```python
from build123d import *

# Parameters (mm, degrees)
HEX_BODY_9AF_DEPTH            = 2.5
COLLAR_7_5_SKETCH_R           = 3.75
COLLAR_7_5_DEPTH              = 2
TIP_BODY_5_5_SKETCH_R         = 2.75
TIP_BODY_5_5_DEPTH            = 5
TIP_END_CHAMFER_0_5X30_SIZE   = 0.5
TIP_END_CHAMFER_0_5X30_SIZE2  = 0.288675135
TIP_BORE_2_5_SKETCH_R         = 1.25
TIP_BORE_2_5_DEPTH            = 4
SHANK_START                   = 3
SHANK_7_5_SKETCH_R            = 3.75
SHANK_7_5_DEPTH               = 3
SHANK_CHAMFER_1X45_SIZE       = 1
TERMINAL_NOTCH_CUT_DEPTH      = 12.7260394
TERMINAL_NOTCH_CUT_DEPTH_BACK = 12.7260394


with BuildPart() as part:
    # Hex Profile 9AF Sketch → Hex Body 9AF (new body)
    with BuildSketch(Plane.XY):
        Polygon((2.598076211, 4.5), (-2.598076211, 4.5), (-5.196152423, 0), (-2.598076211, -4.5), (2.598076211, -4.5), (5.196152423, 0), align=None)
    extrude(amount=HEX_BODY_9AF_DEPTH)

    # Collar Ø7.5 Sketch → Collar Ø7.5 (add)
    with BuildSketch(Plane.XY.offset(2.5)):
        Circle(COLLAR_7_5_SKETCH_R)
    extrude(amount=COLLAR_7_5_DEPTH)

    # Tip Body Ø5.5 Sketch → Tip Body Ø5.5 (add)
    with BuildSketch(Plane.XY.offset(4.5)):
        Circle(TIP_BODY_5_5_SKETCH_R)
    extrude(amount=TIP_BODY_5_5_DEPTH)

    # Tip End Chamfer 0.5x30
    tip_end_chamfer_0_5x30_edges = [part.edges().sort_by_distance(p)[0] for p in [
        (-2.75, 0, 9.5),
    ]]
    tip_end_chamfer_0_5x30_side = [part.faces().sort_by_distance(p)[0] for p in [
        (-2.75, 0, 7),
    ]]
    chamfer(tip_end_chamfer_0_5x30_edges, length=TIP_END_CHAMFER_0_5X30_SIZE, length2=TIP_END_CHAMFER_0_5X30_SIZE2, reference=tip_end_chamfer_0_5x30_side[0])

    # Tip Bore Ø2.5 Sketch → Tip Bore Ø2.5 (cut)
    with BuildSketch(Plane.XY.offset(9.5)):
        Circle(TIP_BORE_2_5_SKETCH_R)
    extrude(amount=-TIP_BORE_2_5_DEPTH, mode=Mode.SUBTRACT)

    # Shank Ø7.5 Sketch → Shank Ø7.5 (add)
    with BuildSketch(Plane(origin=(0, 0, 0), x_dir=(-1, 0, 0), z_dir=(0, 0, -1)).offset(SHANK_START)):
        with Locations(Location((0, 0, 0), (0, 0, 180))):
            Circle(SHANK_7_5_SKETCH_R)
    extrude(amount=-SHANK_7_5_DEPTH)

    # Shank Chamfer 1x45
    shank_chamfer_1x45_edges = [part.edges().sort_by_distance(p)[0] for p in [
        (-3.75, 0, -3),
    ]]
    chamfer(shank_chamfer_1x45_edges, length=SHANK_CHAMFER_1X45_SIZE)

    # Terminal Stud Profile Sketch → Terminal Stud (revolve)
    with BuildSketch(Plane(origin=(0, 0, 0), x_dir=(0, 0, -1), z_dir=(1, 0, 0)), mode=Mode.PRIVATE) as terminal_stud_sk:
        Polygon((3, -1.245), (4.5, -1.245), (4.5, -0.995), (5, -0.995), (5, -1.245), (5.5, -1.245), (5.5, -0.995), (6, -0.995), (6, 0), (3, 0), align=None)
    revolve(terminal_stud_sk.sketch.rotate(Axis((0, 0, -3), (0, 0, -1)), 270), axis=Axis((0, 0, -3), (0, 0, -1)))

    # Terminal Notch Sketch → Terminal Notch Cut (cut, two sides: drawn at the far end of the back side and taken through both)
    with BuildSketch(Plane(origin=(0, 0, 0), x_dir=(0, 0, -1), z_dir=(1, 0, 0)).offset(-TERMINAL_NOTCH_CUT_DEPTH_BACK)):
        Polygon((6, 0.695), (5.7, 0.995), (6, 0.995), align=None)
    extrude(amount=TERMINAL_NOTCH_CUT_DEPTH + TERMINAL_NOTCH_CUT_DEPTH_BACK, mode=Mode.SUBTRACT)


solid = part.part
```
Verification items for the finished model (mm, model axes). A direction names the side the tool comes from. Round coordinates to 2 decimals unless told otherwise and drop trailing zeros. Write each loop counter-clockwise with the first axis right and the second up, starting at its lowest first coordinate (ties: lowest second). Pieces come first, ordered by that corner, then holes. Notation, with made-up numbers: (-1, -5.5) - (21, -5.5) arc R24 cw to (21, 32.5) - close; hole circle Ø5 at (73.25, 17.5). An arc over 180 degrees is marked (long way). Answer as a JSON object with one key per item and string values. Group by question number.
Q1. Tool access check on faces 4 (the cylindrical face through (1.19, -0.37, -5.25)), 5 (the cylindrical face through (-3.746, 0.165, 3.486)), 6 (the flat face through (3.88, -2.28, 1.23)). Record the directions out of +Z, -Z, +X, -X, +Y, -Y that give a thin tool (end or side, any length) a straight path to the whole face; none if there is none.
Q2. Thickness scan on line 1 (Y direction, x = 0, z = 6.9); line 2 (Z direction, x = -3, y = -3); line 3 (Z direction, x = -0.5, y = -2.25). Record the ranges inside material, lowest first.
Q3. Section check A-A, the plane z = 2. Enter the section's corners in (x, y), plus the area to 3 significant figures.
Q4. Go/stop test with flat-tipped pins: pin 1 Ø1.5 at (x, z) = (0.5, 4) entering from +Y; pin 2 Ø0.8 at (x, y) = (-0.5, 0) entering from +Z; pin 3 Ø1.5 at (y, z) = (3, -4) entering from -X; pin 4 Ø1.5 at (y, z) = (2.5, 5) entering from +X. Record where each tip stops, or that it passes through.
Q5. Section check B-B, the plane z = -2.75. Enter the section's corners in (x, y).
Q6. Mould release check, pull along X, two halves, no side actions. Record for faces 1 (the flat face through (1, 4, 0)), 2 (the flat face through (0, 0, 5.5)), 3 (the flat face through (-3.88, 2.28, 1.23)): released by +X, released by -X, zero draft, split by the parting line, or undercut.
Found:
{
 "1": {"face 4": "-Z", "face 5": "+Z", "face 6": "+Z, -Z, +X, -Y"},
 "2": {"line 1": "y = -2.75 to -1.25, 1.25 to 2.75", "line 2": "z = 0 to 2.5", "line 3": "z = -3 to 9.5"},
 "3": {"outline": "(-5.2, 0) - (-2.6, -4.5) - (2.6, -4.5) - (5.2, 0) - (2.6, 4.5) - (-2.6, 4.5) - close", "area": "70.1 mm^2"},
 "4": {"pin 1": "stops at y = 3.75", "pin 2": "stops at z = 5.5", "pin 3": "passes through", "pin 4": "stops at x = 3.21"},
 "5": {"outline": "circle Ø6 at (0, 0)"},
 "6": {"face 1": "zero draft", "face 2": "undercut", "face 3": "released by -X"}
}
